Geometry check sheet. Reference: the model listing, model coordinates, mm. A direction names the side the tool comes from. Give positions to 0.01 mm unless a question says otherwise; leave off trailing zeros. Order: outer loops, then holes, each group sorted by start corner. A loop starts at its lowest first (then second) coordinate and runs counter-clockwise, first axis right, second up.
from build123d import *

# Parameters (mm, degrees)
BOSS_EXTRUDE1_DEPTH = 2.8
SKETCH3_W           = 4.45
SKETCH3_H           = 4.3
BOSS_EXTRUDE2_DEPTH = 1.5
SKETCH4_R           = 4.5
CUT_EXTRUDE2_DEPTH  = 10
BOSS_EXTRUDE3_DEPTH = 1.5
CUT_EXTRUDE5_DEPTH  = 12.445086282
SKETCH17_W          = 15
SKETCH17_H          = 30
BOSS_EXTRUDE4_DEPTH = 3
CUT_EXTRUDE6_DEPTH  = 233


with BuildPart() as part:
    # Sketch1 → Boss-Extrude1 (new body)
    with BuildSketch(Plane(origin=(0, 0, 0), x_dir=(1, 0, 0), z_dir=(0, 1, 0))):
        with BuildLine():
            Line((-3.05, 0), (-3.05, 7.5))
            Line((-3.05, 7.5), (-7.5, 7.5))
            Line((-7.5, 7.5), (-7.5, -7.5))
            Line((-7.5, -7.5), (7.5, -7.5))
            Line((7.5, -7.5), (7.5, 7.5))
            Line((7.5, 7.5), (3.05, 7.5))
            Line((3.05, 7.5), (3.05, 0))
            ThreePointArc((3.05, 0), (0, -3.05), (-3.05, 0))
        make_face()
    extrude(amount=BOSS_EXTRUDE1_DEPTH)

    # Sketch3 → Boss-Extrude2 (add)
    with BuildSketch(Plane(origin=(0, 2.8, 0), x_dir=(1, 0, 0), z_dir=(0, 1, 0))):
        with Locations((-5.275, 5.35)):
            Rectangle(SKETCH3_W, SKETCH3_H)
        with Locations((5.275, 5.35)):
            Rectangle(SKETCH3_W, SKETCH3_H)
    extrude(amount=BOSS_EXTRUDE2_DEPTH)

    # Sketch4 → Cut-Extrude2 (cut)
    with BuildSketch(Plane(origin=(0, 2.8, 0), x_dir=(1, 0, 0), z_dir=(0, 1, 0))):
        Circle(SKETCH4_R)
    extrude(amount=CUT_EXTRUDE2_DEPTH, mode=Mode.SUBTRACT)

    # Sketch5 → Boss-Extrude3 (add)
    with BuildSketch(Plane(origin=(0, 2.8, 0), x_dir=(1, 0, 0), z_dir=(0, 1, 0))):
        with BuildLine():
            Line((-7.5, 3.2), (-7.5, 0))
            Line((-7.5, 0), (-4.5, 0))
            ThreePointArc((-4.5, 0), (-4.152551193, 1.733873868), (-3.163858404, 3.2))
            Line((-3.163858404, 3.2), (-7.5, 3.2))
        make_face()
        with BuildLine():
            ThreePointArc((3.163858404, 3.2), (4.152551193, 1.733873868), (4.5, 0))
            Line((4.5, 0), (7.5, 0))
            Line((7.5, 0), (7.5, 3.2))
            Line((7.5, 3.2), (3.163858404, 3.2))
        make_face()
    extrude(amount=BOSS_EXTRUDE3_DEPTH)

    # Sketch14 → Cut-Extrude5 (cut, through all)
    with BuildSketch(Plane(origin=(0, 4.3, 0), x_dir=(1, 0, 0), z_dir=(0, 1, 0))):
        Polygon((4.5, 7.5), (7.5, 4.5), (7.5, 7.5), align=None)
        Polygon((-7.5, 7.5), (-4.5, 7.5), (-7.5, 4.5), align=None)
    extrude(amount=-CUT_EXTRUDE5_DEPTH, mode=Mode.SUBTRACT)

    # Sketch16 → M2 Tapped Hole1 (revolve, cut)
    with BuildSketch(Plane(origin=(5.914213562, 1.4, -6.085786438), x_dir=(-0.7071067811865475, 0, -0.7071067811865477), z_dir=(0, 1, 0))):
        Polygon((0, 0), (0, 8.480688495), (0.8, 8), (0.8, 0), align=None)
    m2_tapped_hole1 = revolve(axis=Axis((10.404341623, 1.4, -10.575914498), (-0.7071067811865477, 0, 0.7071067811865475)), mode=Mode.SUBTRACT)

    # Mirror1: M2 Tapped Hole1 across plane
    add(m2_tapped_hole1.mirror(Plane(origin=(0, 0, 0), x_dir=(0, 0, 1), z_dir=(1, 0, 0))), mode=Mode.SUBTRACT)

    # Sketch17 → Boss-Extrude4 (add)
    with BuildSketch(Plane.XY.offset(7.5)):
        with Locations((0, -12.2)):
            Rectangle(SKETCH17_W, SKETCH17_H)
    extrude(amount=BOSS_EXTRUDE4_DEPTH)

    # Sketch18 → Cut-Extrude6 (cut)
    with BuildSketch(Plane(origin=(0, 0, 7.5), x_dir=(-1, 0, 0), z_dir=(0, 0, -1))):
        with BuildLine():
            Line((-1.6, -27.2), (-1.6, -2.2))
            ThreePointArc((-1.6, -2.2), (0, -0.6), (1.6, -2.2))
            Line((1.6, -2.2), (1.6, -27.2))
            ThreePointArc((1.6, -27.2), (0, -28.8), (-1.6, -27.2))
        make_face()
    extrude(amount=-CUT_EXTRUDE6_DEPTH, mode=Mode.SUBTRACT)


solid = part.part
Item 1: Gauge pin test, flat ends, axial feed: pin 1 (1 mm diameter, centred on x = 4, z = -3.5, fed in from -Y); pin 2 (1.5 mm diameter, centred on x = -6, y = -15.5, fed in from -Z); pin 3 (7 mm diameter, centred on x = 1.5, z = 2.5, fed in from +Y). Record the tip position at first contact, or that the pin passes through.
Reported:
pin 1: stops at y = 0
pin 2: stops at z = 7.5
pin 3: stops at y = 2.8
Item 2: Set-up check for faces 1 (the flat face through (-3.05, 2, -5)), 2 (the flat face through (-1.6, -15, 9)), 3 (the flat face through (-6, 4, 0)): record each of +Z, -Z, +X, -X, +Y, -Y from which the full face is reachable in a straight line by a thin tool's end or side.
Reported:
face 1: -Z, +Y, -Y
face 2: +Z, -Z, -Y
face 3: +Z, +X, -X, +Y
Item 3: Draft check along Z on faces 4 (the cylindrical face through (5.15, 1.36, -4.19)), 5 (the flat face through (-2, -13, 7.5)), 6 (the flat face through (-5, 4.3, -4)). Enter one of: released by +Z, released by -Z, zero draft, split by the parting line, or undercut.
Reported:
face 4: undercut
face 5: released by -Z
face 6: zero draft
Item 4: Sectioned sample at C-C (x = 0). Enter the section's corners in (y, z), and give its area (3 significant figures).
Reported:
outline: (-0.6, 7.5) - (0, 7.5) - (0, 3.05) - (2.8, 3.05) - (2.8, 10.5) - (-0.6, 10.5) - close
area: 22.7 mm2
Item 5: Sectioned sample at D-D (z = -1.75). Enter the section's corners in (x, y), and give its area (3 significant figures).
Reported:
outline: (-7.5, 0) - (-3.05, 0) - (-3.05, 2.8) - (-4.15, 2.8) - (-4.15, 4.3) - (-7.5, 4.3) - close; (3.05, 0) - (7.5, 0) - (7.5, 4.3) - (4.15, 4.3) - (4.15, 2.8) - (3.05, 2.8) - close
area: 35.0 mm2
Item 6: Sectioned sample at B-B (z = 1). Enter the section's corners in (x, y), and give its area (3 significant figures).
Reported:
outline: (-7.5, 0) - (-2.88, 0) - (-2.88, 2.8) - (-7.5, 2.8) - close; (2.88, 0) - (7.5, 0) - (7.5, 2.8) - (2.88, 2.8) - close
area: 25.9 mm2
Item 7: Scan lines: L1, parallel to X at y = -21.5, z = 9.5; L2, parallel to Z at x = 4.25, y = -7.5; L3, parallel to Y at x = 3, z = 4.75. Record each from-to range of solid material in increasing order.
Reported:
L1: x = -7.5 to -1.6, 1.6 to 7.5
L2: z = 7.5 to 10.5
L3: y = 0 to 2.8
Item 8: Sectioned sample at A-A (y = -23.5). Enter the section's corners in (x, z).
Reported:
outline: (-7.5, 7.5) - (-1.6, 7.5) - (-1.6, 10.5) - (-7.5, 10.5) - close; (1.6, 7.5) - (7.5, 7.5) - (7.5, 10.5) - (1.6, 10.5) - close
